Read the model definition and answer for the solid it produces. Units are mm, in the model's axes. Round coordinates to 2 decimals unless told otherwise and drop trailing zeros. Order: outer loops, then holes, each group sorted by start corner. A loop starts at its lowest first (then second) coordinate and runs counter-clockwise, first axis right, second up. Notation, with made-up numbers: M 19.5,-3.75 L 27.5,-3.75 A13 ccw 27.5,16.25 Z; hole C 66.5,26.25 d1. An arc over 180 degrees is marked long. Use one line per item in the form item = value. Start each with the question number.
from build123d import *

# Parameters (mm, degrees)
SKETCH1_R           = 5.2
BOSS_EXTRUDE1_DEPTH = 8


with BuildPart() as part:
    # Sketch1 → Boss-Extrude1 (new body)
    with BuildSketch(Plane.XY):
        Polygon((0, 9.237604307), (-8, 4.618802154), (-8, -4.618802154), (0, -9.237604307), (8, -4.618802154), (8, 4.618802154), align=None)
        Circle(SKETCH1_R, mode=Mode.SUBTRACT)
    extrude(amount=BOSS_EXTRUDE1_DEPTH)


solid = part.part
Item 1: Section D-D (y = 6) is taken. Write down the section's boundary in (x, z).
Item 2: Section A-A (y = 0) is taken. Write down the section's boundary in (x, z).
Item 3: Section B-B (z = 4.25) is taken. Write down the section's boundary in (x, y).
Item 4: Find the intervals of material crossed by L1, parallel to Y at x = 4, z = 6.75; L2, parallel to Y at x = 3.25, z = 1.75; L3, parallel to X at y = 0.5, z = 3, in increasing order. Write a range as [from, to].
Item 5: Given P1, Ø1.5, axis at x = -4.5, z = 4, coming from the +Y side, flat-ended and moving along its own axis, determine where the tip first touches the part or whether it passes through.
Item 6: For a pull along X with two mould halves and no side action, classify faces 1 (the flat face through (-3.944, 6.961, 3.944)), 2 (the flat face through (3.944, -6.961, 3.944)), 3 (the cylindrical face through (-0.677, 5.156, 3.944)) as pulls with the +X half, pulls with the -X half, needs draft (parallel to the pull), parting line crosses it, or undercut.
Item 7: Section C-C (x = -1) is taken. Write down the section's boundary in (y, z), and give its area (3 significant figures).
The answers:
q1.outline = M -5.61,0 L 5.61,0 L 5.61,8 L -5.61,8 Z
q2.outline = M -8,0 L -5.2,0 L -5.2,8 L -8,8 Z; M 5.2,0 L 8,0 L 8,8 L 5.2,8 Z
q3.outline = M -8,-4.62 L 0,-9.24 L 8,-4.62 L 8,4.62 L 0,9.24 L -8,4.62 Z; hole C 0,0 d10.4
q4.L1 = [-6.93, -3.32], [3.32, 6.93]
q4.L2 = [-7.36, -4.06], [4.06, 7.36]
q4.L3 = [-8, -5.18], [5.18, 8]
q5.P1 = 7.07
q6.face_1 = pulls with the -X half
q6.face_2 = pulls with the +X half
q6.face_3 = undercut
q7.outline = M -8.66,0 L -5.1,0 L -5.1,8 L -8.66,8 Z; M 5.1,0 L 8.66,0 L 8.66,8 L 5.1,8 Z
q7.area = 56.9 mm²
